```python
from build123d import *

# Parameters (mm, degrees)
BRACKET_L_PROFILE_SKETCH_W                   = 100
BRACKET_L_PROFILE_SKETCH_H                   = 80
BRACKET_BODY_DEPTH                           = 125
RECTANGULAR_CUT_SKETCH_10X15_W               = 85
RECTANGULAR_CUT_SKETCH_10X15_H               = 70
RECTANGULAR_CUT_10X15_DEPTH                  = 100
COUNTERSUNK_HOLES_6XM6_D                     = 6.6
COUNTERSUNK_HOLES_6XM6_DEPTH                 = 36.017159957
COUNTERSUNK_HOLES_6XM6_CSINK_D               = 12.6
COUNTERSUNK_HOLES_6XM6_CSINK_ANGLE           = 90
COUNTERSUNK_HOLES_6XM6_TIP                   = 1.982840043
COUNTERSUNK_HOLES_6XM6_ON_FACE_2_D           = 6.6
COUNTERSUNK_HOLES_6XM6_ON_FACE_2_DEPTH       = 36.017159957
COUNTERSUNK_HOLES_6XM6_ON_FACE_2_CSINK_D     = 12.6
COUNTERSUNK_HOLES_6XM6_ON_FACE_2_CSINK_ANGLE = 90
COUNTERSUNK_HOLES_6XM6_ON_FACE_2_TIP         = 1.982840043
COUNTERSUNK_HOLES_6XM6_ON_FACE_3_D           = 6.6
COUNTERSUNK_HOLES_6XM6_ON_FACE_3_DEPTH       = 36.017159957
COUNTERSUNK_HOLES_6XM6_ON_FACE_3_CSINK_D     = 12.6
COUNTERSUNK_HOLES_6XM6_ON_FACE_3_CSINK_ANGLE = 90
COUNTERSUNK_HOLES_6XM6_ON_FACE_3_TIP         = 1.982840043
OUTER_EDGE_FILLETS_R10_R                     = 10
EDGE_FILLETS_R2_R                            = 2


with BuildPart() as part:
    # Bracket L-Profile Sketch → Bracket Body (new body)
    with BuildSketch(Plane.XY):
        Rectangle(BRACKET_L_PROFILE_SKETCH_W, BRACKET_L_PROFILE_SKETCH_H)
    extrude(amount=BRACKET_BODY_DEPTH)

    # Rectangular Cut Sketch 10x15 → Rectangular Cut 10x15 (cut)
    with BuildSketch(Plane.XY.offset(125)):
        with Locations((7.5, 5)):
            Rectangle(RECTANGULAR_CUT_SKETCH_10X15_W, RECTANGULAR_CUT_SKETCH_10X15_H)
    extrude(amount=-RECTANGULAR_CUT_10X15_DEPTH, mode=Mode.SUBTRACT)

    # Countersunk Holes 6xM6
    with Locations(Plane(origin=(-35, -5, 100), x_dir=(0, 1, 0), z_dir=(1, 0, 0))):
        with Locations((0, 0), (20, -50)):
            CounterSinkHole(COUNTERSUNK_HOLES_6XM6_D / 2, COUNTERSUNK_HOLES_6XM6_CSINK_D / 2, depth=COUNTERSUNK_HOLES_6XM6_DEPTH, counter_sink_angle=COUNTERSUNK_HOLES_6XM6_CSINK_ANGLE)
            with Locations((0, 0, -(COUNTERSUNK_HOLES_6XM6_DEPTH + COUNTERSUNK_HOLES_6XM6_TIP / 2))):  # 118° drill point
                Cone(0, COUNTERSUNK_HOLES_6XM6_D / 2, COUNTERSUNK_HOLES_6XM6_TIP, mode=Mode.SUBTRACT)

    # Countersunk Holes 6xM6 on face 2
    with Locations(Plane(origin=(-10, -30, 100), x_dir=(0, 0, 1), z_dir=(0, 1, 0))):
        with Locations((0, 0), (-50, 35)):
            CounterSinkHole(COUNTERSUNK_HOLES_6XM6_ON_FACE_2_D / 2, COUNTERSUNK_HOLES_6XM6_ON_FACE_2_CSINK_D / 2, depth=COUNTERSUNK_HOLES_6XM6_ON_FACE_2_DEPTH, counter_sink_angle=COUNTERSUNK_HOLES_6XM6_ON_FACE_2_CSINK_ANGLE)
            with Locations((0, 0, -(COUNTERSUNK_HOLES_6XM6_ON_FACE_2_DEPTH + COUNTERSUNK_HOLES_6XM6_ON_FACE_2_TIP / 2))):  # 118° drill point
                Cone(0, COUNTERSUNK_HOLES_6XM6_ON_FACE_2_D / 2, COUNTERSUNK_HOLES_6XM6_ON_FACE_2_TIP, mode=Mode.SUBTRACT)

    # Countersunk Holes 6xM6 on face 3
    with Locations(Plane(origin=(25, -5, 25), x_dir=(1, 0, 0), z_dir=(0, 0, 1))):
        with Locations((0, 0), (-35, 20)):
            CounterSinkHole(COUNTERSUNK_HOLES_6XM6_ON_FACE_3_D / 2, COUNTERSUNK_HOLES_6XM6_ON_FACE_3_CSINK_D / 2, depth=COUNTERSUNK_HOLES_6XM6_ON_FACE_3_DEPTH, counter_sink_angle=COUNTERSUNK_HOLES_6XM6_ON_FACE_3_CSINK_ANGLE)
            with Locations((0, 0, -(COUNTERSUNK_HOLES_6XM6_ON_FACE_3_DEPTH + COUNTERSUNK_HOLES_6XM6_ON_FACE_3_TIP / 2))):  # 118° drill point
                Cone(0, COUNTERSUNK_HOLES_6XM6_ON_FACE_3_D / 2, COUNTERSUNK_HOLES_6XM6_ON_FACE_3_TIP, mode=Mode.SUBTRACT)

    # Outer Edge Fillets R10
    outer_edge_fillets_r10_edges = [part.edges().sort_by_distance(p)[0] for p in [
        (50, -35, 125),
        (-42.5, 40, 125),
        (50, 40, 12.5),
        (0, 40, 0),
        (50, 0, 0),
        (0, -40, 0),
        (-50, 0, 0),
        (-50, -40, 62.5),
    ]]
    fillet(outer_edge_fillets_r10_edges, radius=OUTER_EDGE_FILLETS_R10_R)

    # Edge Fillets R2
    edge_fillets_r2_edges = [part.edges().sort_by_distance(p)[0] for p in [
        (-35, 5, 25),
        (-35, -30, 75),
        (7.5, -30, 25),
    ]]
    fillet(edge_fillets_r2_edges, radius=EDGE_FILLETS_R2_R)


solid = part.part
```
Source: CAD feature listing. Evaluate the final solid. Frame: model axes, mm. A direction names the side the tool comes from. Coordinates: 2 decimals unless noted, no trailing zeros. Write each loop counter-clockwise with the first axis right and the second up, starting at its lowest first coordinate (ties: lowest second). Pieces come first, ordered by that corner, then holes. Notation, with made-up numbers: (63.5, 24) -> (78.5, 24) arc R19 ccw to (78.5, 29) -> close; hole circle Ø6 at (56, -33.5). An arc over 180 degrees is marked (long way). Return JSON: item names as keys, results as strings. Group by question number.
1) Contact query for flat-ended pins moving along their axis: P1, Ø10.5, axis at x = -10, z = 100, coming from the +Y side; P2, Ø10.5, axis at y = -5, z = 100, coming from the -X side; P3, Ø12, axis at x = 10.5, z = 35, coming from the +Y side; P4, Ø5, axis at x = 21.5, z = 28.5, coming from the +Y side. Output: stop coordinate, or through.
2) Section query D-D, the plane y = -21. Return loops of the section in (x, z).
3) Section query C-C, the plane y = 15. Return loops of the section in (x, z), plus the area to 3 significant figures.
4) Section query A-A, the plane z = 100. Return loops of the section in (x, y).
5) Section query B-B, the plane x = -10. Return loops of the section in (y, z).
6) Mould query, pull axis X, two halves, no side actions, for faces 3 (the face through (50, -31, 39)), 4 (the face through (-47.15, -36.99, 68.3)), 5 (the face through (-42.4, 37.15, 121.99)), 6 (the face through (-7.266, 12.903, 22.146)). Classes: +X half, -X half, draft (parallel to the pull), parting line (faces both ways), or undercut.
7) Set-up query: faces 1 (the face through (22.992, -36.549, 52.619)), 2 (the face through (-35, 6, 77)). Return all of +Z, -Z, +X, -X, +Y, -Y with unobstructed straight access to the full face (end or side cutting, diameter ignored); none if empty.
8) Ray query, line 1 along Y through (x, z) = (25, 11.75); line 2 along X through (y, z) = (15, 14); line 3 along X through (y, z) = (1.5, 31.5). Return the intervals inside material, ascending.
From the geometry:
{
 "1": {"P1": "y = -31.05", "P2": "x = -50", "P3": "y = -30", "P4": "y = -29.73"},
 "2": {"outline": "(-50, 10) arc R10 ccw to (-40, 0) -> (40, 0) arc R10 ccw to (50, 10) -> (50, 25) -> (-33, 25) arc R2 cw to (-35, 27) -> (-35, 125) -> (-50, 125) -> close"},
 "3": {"outline": "(-50, 10) arc R10 ccw to (-40, 0) -> (-13.3, 0) -> (-13.3, 22) -> (-16.3, 25) -> (-33, 25) arc R2 cw to (-35, 27) -> (-35, 43.7) -> (-38, 46.7) -> (-50, 46.7) -> close; (-50, 53.3) -> (-38, 53.3) -> (-35, 56.3) -> (-35, 125) -> (-50, 125) -> close; (-6.7, 0) -> (40, 0) arc R10 ccw to (50, 10) -> (50, 25) -> (-3.7, 25) -> (-6.7, 22) -> close", "area": "3,680 mm²"},
 "4": {"outline": "(-50, -30) arc R10 ccw to (-40, -40) -> (-13.3, -40) -> (-13.3, -33) -> (-16.3, -30) -> (-33, -30) arc R2 cw to (-35, -28) -> (-35, -11.3) -> (-38, -8.3) -> (-50, -8.3) -> close; (-50, -1.7) -> (-38, -1.7) -> (-35, 1.3) -> (-35, 40) -> (-50, 40) -> close; (-6.7, -40) -> (50, -40) -> (50, -30) -> (-3.7, -30) -> (-6.7, -33) -> close"},
 "5": {"outline": "(-40, 10) arc R10 ccw to (-30, 0) -> (11.7, 0) -> (11.7, 22) -> (8.7, 25) -> (-28, 25) arc R2 cw to (-30, 27) -> (-30, 93.7) -> (-33, 96.7) -> (-40, 96.7) -> close; (-40, 103.3) -> (-33, 103.3) -> (-30, 106.3) -> (-30, 125) -> (-40, 125) -> close; (18.3, 0) -> (30, 0) arc R10 ccw to (40, 10) -> (40, 25) -> (21.3, 25) -> (18.3, 22) -> close"},
 "6": {"face 3": "+X half", "face 4": "-X half", "face 5": "draft", "face 6": "undercut"},
 "7": {"face 1": "+Y, -Y", "face 2": "+Z, +X, +Y"},
 "8": {"line 1": "-40 to -8.3, -1.7 to 40", "line 2": "-50 to -13.3, -6.7 to 50", "line 3": "-50 to -35"}
}
